The model under review builds one solid part; all positions refer to its coordinate system, in mm. Face numbers are marked on the shaded views. A direction names the side the tool comes from. Coordinates: 2 decimals unless noted, no trailing zeros. Order: outer loops, then holes, each group sorted by start corner. A loop starts at its lowest first (then second) coordinate and runs counter-clockwise, first axis right, second up. Notation, with made-up numbers: (-16, 56.25) - (34, 56.25) arc R23 cw to (34, 81.25) - close; hole circle Ø4 at (24, 3.25). An arc over 180 degrees is marked (long way). Answer in a Markdown table with one row per item.
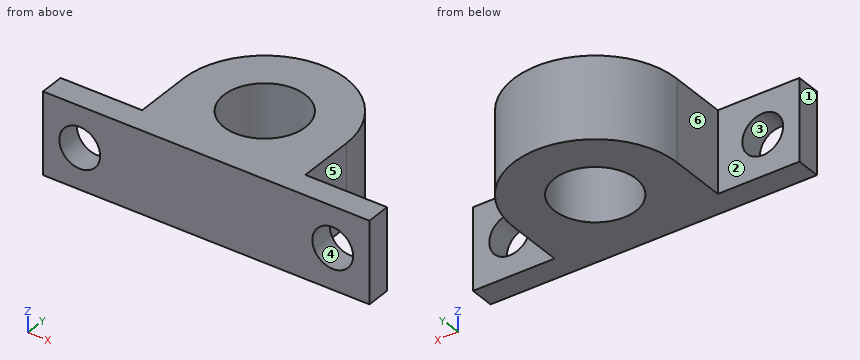
```python
from build123d import *

# Parameters (mm, degrees)
SKETCH1_R           = 10
BOSS_EXTRUDE1_DEPTH = 10
SKETCH2_R           = 5
CUT_EXTRUDE1_DEPTH  = 10


with BuildPart() as part:
    # Sketch1 → Boss-Extrude1 (new, symmetric)
    with BuildSketch(Plane.XY):
        with BuildLine():
            Line((-40, -14), (-40, -20))
            Line((-40, -20), (40, -20))
            Line((40, -20), (40, -14))
            Line((40, -14), (20, -14))
            Line((20, -14), (20, 0))
            ThreePointArc((20, 0), (0, 20), (-20, 0))
            Line((-20, 0), (-20, -14))
            Line((-20, -14), (-40, -14))
        make_face()
        Circle(SKETCH1_R, mode=Mode.SUBTRACT)
    extrude(amount=BOSS_EXTRUDE1_DEPTH, both=True)

    # Sketch2 → Cut-Extrude1 (cut, symmetric)
    with BuildSketch(Plane(origin=(0, -14, 0), x_dir=(1, 0, 0), z_dir=(0, 1, 0))):
        with Locations(Location((31, 0, 0), (0, 0, 180))):
            Circle(SKETCH2_R)
        with Locations(Location((-31, 0, 0), (0, 0, 180))):
            Circle(SKETCH2_R)
    extrude(amount=CUT_EXTRUDE1_DEPTH, both=True, mode=Mode.SUBTRACT)


solid = part.part
```
Item 1: Mouldability with a two-part tool opening along X and no side actions: class the marked faces 1, 2 and 3 as +X half, -X half, draft (parallel to the pull), parting line (faces both ways), or undercut.
Check values:
| item | result |
|---|---|
| face 1 | -X half |
| face 2 | draft |
| face 3 | undercut |
Item 2: We need section B-B, the plane x = 0. Write out the cut boundary in (y, z).
Check values:
| item | result |
|---|---|
| outline | (-20, -10) - (-10, -10) - (-10, 10) - (-20, 10) - close; (10, -10) - (20, -10) - (20, 10) - (10, 10) - close |
Item 3: We need section D-D, the plane z = -6.25. Write out the cut boundary in (x, y), then the cut area to 3 significant figures.
Check values:
| item | result |
|---|---|
| outline | (-40, -20) - (40, -20) - (40, -14) - (20, -14) - (20, 0) arc R20 ccw to (-20, 0) - (-20, -14) - (-40, -14) - close; hole circle Ø20 at (0, 0) |
| area | 1,350 mm^2 |
Item 4: We need section A-A, the plane z = 0. Write out the cut boundary in (x, y), then the cut area to 3 significant figures.
Check values:
| item | result |
|---|---|
| outline | (-40, -20) - (-36, -20) - (-36, -14) - (-40, -14) - close; (-26, -20) - (26, -20) - (26, -14) - (20, -14) - (20, 0) arc R20 ccw to (-20, 0) - (-20, -14) - (-26, -14) - close; (36, -20) - (40, -20) - (40, -14) - (36, -14) - close; hole circle Ø20 at (0, 0) |
| area | 1,230 mm^2 |
Item 5: Clearance check with flat-ended pins moving along their axes: pin 1 Ø6 at (x, z) = (-30.5, -5) entering from +Y; pin 2 Ø1.5 at (x, z) = (1, -3.5) entering from +Y; pin 3 Ø1 at (y, z) = (7, 3.5) entering from -X. State where each tip first meets the part, or that it passes through.
Check values:
| item | result |
|---|---|
| pin 1 | y = -14 |
| pin 2 | y = 20 |
| pin 3 | x = -18.91 |
Item 6: Tool access review of the marked faces 4, 5 and 6: name each direction out of +Z, -Z, +X, -X, +Y, -Y from which nothing blocks a thin tool from reaching the whole face with its end or side.
Check values:
| item | result |
|---|---|
| face 4 | +Y, -Y |
| face 5 | +Z, -Z, +X, +Y |
| face 6 | +Z, -Z, -X, +Y |
Item 7: To check wall thickness, follow line 1 (Z direction, x = -31, y = -17.1); line 2 (X direction, y = -8, z = -2); line 3 (Y direction, x = 28, z = -8.25). State the ranges of each line that lie inside material, in increasing order. Write a range as from..to.
Check values:
| item | result |
|---|---|
| line 1 | -10..-5, 5..10 |
| line 2 | -20..-6, 6..20 |
| line 3 | -20..-14 |
Item 8: We need section C-C, the plane y = -16. Write out the cut boundary in (x, z).
Check values:
| item | result |
|---|---|
| outline | (-40, -10) - (40, -10) - (40, 10) - (-40, 10) - close; hole circle Ø10 at (-31, 0); hole circle Ø10 at (31, 0) |
